Build history of the part. All positions in model axes, mm. A direction names the side the tool comes from. Coordinates: 2 decimals unless noted, no trailing zeros. Loops run counter-clockwise (first coordinate to the right, second up) from the corner with the lowest first, then second, coordinate; pieces in that order, holes last. Notation, with made-up numbers: M 5,48 L 58,48 A22 cw 58,74 Z; hole C 89.25,-1 d9. An arc over 180 degrees is marked long. Write each question's results on one line, items separated by ' | '. Start each with the question number.
from build123d import *

# Parameters (mm, degrees)
SKETCH_1_W               = 1457
SKETCH_1_H               = 210
EXTRUDE_1_DEPTH          = 30
SHELL_1_T                = -2
SKETCH_2_W               = 1457
SKETCH_2_H               = 20
EXTRUDE_2_DEPTH          = 2
SKETCH_3_R               = 4.5
CUT_EXTRUDE_1_DEPTH      = 10
CUT_EXTRUDE_2_DEPTH      = 1525
CUT_EXTRUDE_2_DEPTH_BACK = 76
SKETCH_4_R               = 4.5


with BuildPart() as part:
    # 草图1 → 凸台-拉伸1 (new body)
    with BuildSketch(Plane.XY):
        with Locations((728.5, 105)):
            Rectangle(SKETCH_1_W, SKETCH_1_H)
    extrude(amount=EXTRUDE_1_DEPTH)

    # 抽壳1
    shell_1_openings = [part.faces().sort_by_distance(p)[0] for p in [
        (728.5, 105, 30),
    ]]
    offset(amount=SHELL_1_T, openings=shell_1_openings, kind=Kind.INTERSECTION)

    # 草图2 → 凸台-拉伸2 (add)
    with BuildSketch(Plane.XY.offset(30)):
        with Locations((728.5, 220)):
            Rectangle(SKETCH_2_W, SKETCH_2_H)
    extrude(amount=-EXTRUDE_2_DEPTH)

    # 草图3 → 切除-拉伸1 (cut)
    with BuildSketch(Plane(origin=(0, 2, 0), x_dir=(1, 0, 0), z_dir=(0, 1, 0))):
        with Locations(Location((1427, -16, 0), (0, 0, 270))):
            Circle(SKETCH_3_R)
        with Locations(Location((728.5, -16, 0), (0, 0, 270))):
            Circle(SKETCH_3_R)
        with Locations(Location((30, -16, 0), (0, 0, 270))):
            Circle(SKETCH_3_R)
    extrude(amount=-CUT_EXTRUDE_1_DEPTH, mode=Mode.SUBTRACT)

    # 草图4 → 切除-拉伸2 (cut, two sides: drawn at the far end of the back side and taken through both)
    with BuildSketch(Plane(origin=(2, 0, 0), x_dir=(0, 0, -1), z_dir=(1, 0, 0)).offset(-CUT_EXTRUDE_2_DEPTH_BACK)):
        with Locations(Location((-16, 30, 0), (0, 0, 180))):
            Circle(SKETCH_4_R)
        with Locations(Location((-16, 180, 0), (0, 0, 180))):
            Circle(SKETCH_4_R)
    extrude(amount=CUT_EXTRUDE_2_DEPTH + CUT_EXTRUDE_2_DEPTH_BACK, mode=Mode.SUBTRACT)


solid = part.part
1. Wall check: line 1 along X through (y, z) = (0.9, 16); line 2 along X through (y, z) = (84, 4); line 3 along Y through (x, z) = (938, 3). Give the ranges that are in metal, low to high.
2. Band-saw the part on A-A, the plane x = 564. List the corners of the cut face in (y, z), plus the area to 3 significant figures.
3. Pin check, flat tips, straight feed: pin 1 (14 mm diameter, centred on x = 824.5, z = 12, fed in from +Y); pin 2 (12 mm diameter, centred on x = 1172, y = 58, fed in from +Z); pin 3 (8 mm diameter, centred on x = 1427, z = 16, fed in from -Y); pin 4 (8 mm diameter, centred on y = 180, z = 16, fed in from +X). Stop position of each tip, or through.
4. Band-saw the part on B-B, the plane z = 6.5. List the corners of the cut face in (x, y), plus the area to 3 significant figures.
5. Which spindle directions (+Z, -Z, +X, -X, +Y, -Y) get a long thin tool onto all of the face, cutting with end or side? Do faces 5 (the flat face through (718, 106, 0)), 6 (the flat face through (718, 106, 2)). Say none if no direction does.
6. Band-saw the part on C-C, the plane y = 100. List the corners of the cut face in (x, z), plus the area to 3 significant figures.
7. Mould opens along X. For faces 1 (the flat face through (718, 2, 16)), 2 (the flat face through (718, 210, 14)), 3 (the flat face through (0, 113, 15)), 4 (the flat face through (2, 104, 16)) say: +X half, -X half, draft (parallel to the pull), parting line (faces both ways), or undercut.
Checked values:
1) line 1: 0 to 25.5, 34.5 to 724, 733 to 1422.5, 1431.5 to 1457 | line 2: 0 to 2, 1455 to 1457 | line 3: 0 to 2, 208 to 210
2) outline: M 0,0 L 210,0 L 210,28 L 230,28 L 230,30 L 208,30 L 208,2 L 2,2 L 2,30 L 0,30 Z | area: 572 mm²
3) pin 1: y = 210 | pin 2: z = 2 | pin 3: y = 208 | pin 4: through
4) outline: M 0,0 L 1457,0 L 1457,210 L 0,210 Z; hole M 2,2 L 1455,2 L 1455,208 L 2,208 Z | area: 6,650 mm²
5) face 5: -Z, +X, -X, +Y, -Y | face 6: +Z
6) outline: M 0,0 L 1457,0 L 1457,30 L 1455,30 L 1455,2 L 2,2 L 2,30 L 0,30 Z | area: 3,030 mm²
7) face 1: undercut | face 2: draft | face 3: -X half | face 4: undercut
